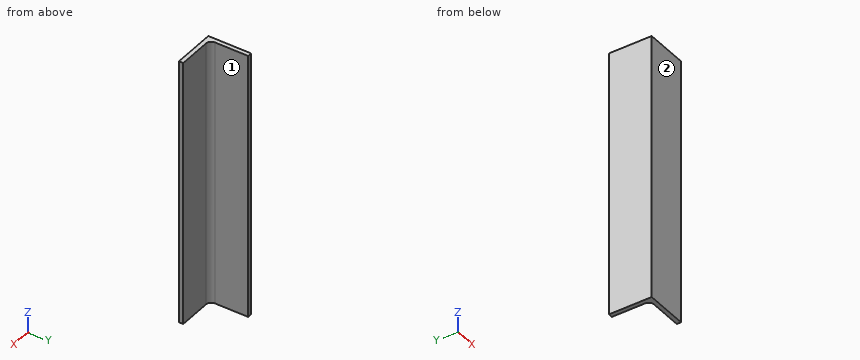
from build123d import *

# Parameters (mm, degrees)
EXTRUDE_1_DEPTH = 250


with BuildPart() as part:
    # 草图1 → 拉伸1 (new body)
    with BuildSketch(Plane.XY):
        with BuildLine():
            Line((0, 0), (0, 40))
            Line((0, 40), (3.99, 40))
            ThreePointArc((3.99, 40), (3.997071068, 39.997071068), (4, 39.99))
            Line((4, 39.99), (4, 9))
            ThreePointArc((4, 9), (5.464466094, 5.464466094), (9, 4))
            Line((9, 4), (39.99, 4))
            ThreePointArc((39.99, 4), (39.997071068, 3.997071068), (40, 3.99))
            Line((40, 3.99), (40, 0))
            Line((40, 0), (0, 0))
        make_face()
    extrude(amount=EXTRUDE_1_DEPTH)


solid = part.part
Geometry: final body of the model. Coordinates: model frame, mm. Face numbers are marked on the shaded views. A direction names the side the tool comes from. Round coordinates to 2 decimals unless told otherwise and drop trailing zeros. Loops run counter-clockwise (first coordinate to the right, second up) from the corner with the lowest first, then second, coordinate; pieces in that order, holes last. Notation, with made-up numbers: M 28.5,15.5 L 35.5,15.5 A21 cw 35.5,42.5 Z; hole C 22,21 d1. An arc over 180 degrees is marked long. Put each result on its own line as item: value. Start each with the question number.
(1) Contact query for flat-ended pins moving along their axis: pin 1 Ø6 at (x, z) = (17.5, 97.5) entering from -Y; pin 2 Ø5 at (x, z) = (24, 206) entering from +Y. Output: stop coordinate, or through.
(2) Material intervals for line 1 along X through (y, z) = (12, 217.5); line 2 along X through (y, z) = (7, 169), sorted ascending. Write a range as [from, to].
(3) Section query B-B (x = 37). Return loops of the section in (y, z).
(4) Set-up query: the marked faces 1 and 2. Return all of +Z, -Z, +X, -X, +Y, -Y with unobstructed straight access to the full face (end or side cutting, diameter ignored); none if empty.
Findings below:
1. pin 1: stops at y = 0
1. pin 2: stops at y = 4
2. line 1: x = [0, 4]
2. line 2: x = [0, 4.42]
3. outline: M 0,0 L 4,0 L 4,250 L 0,250 Z
4. face 1: +Z, -Z, +X, +Y
4. face 2: +Z, -Z, +X, -X, -Y
